```python
from build123d import *

# Parameters (mm, degrees)
SKETCH1_R           = 2
BOSS_EXTRUDE1_DEPTH = 10.8
SKETCH2_R           = 1.7
BOSS_EXTRUDE2_DEPTH = 0.6
SKETCH3_R           = 2
BOSS_EXTRUDE3_DEPTH = 1.6
CHAMFER1_SIZE       = 0.5


with BuildPart() as part:
    # Sketch1 → Boss-Extrude1 (new body)
    with BuildSketch(Plane.XY):
        with Locations(Location((0, 0, 0), (0, 0, 180))):
            Circle(SKETCH1_R)
    extrude(amount=BOSS_EXTRUDE1_DEPTH)

    # Sketch2 → Boss-Extrude2 (add)
    with BuildSketch(Plane.XY.offset(10.8)):
        Circle(SKETCH2_R)
    extrude(amount=BOSS_EXTRUDE2_DEPTH)

    # Sketch3 → Boss-Extrude3 (add)
    with BuildSketch(Plane.XY.offset(11.4)):
        with Locations(Location((0, 0, 0), (0, 0, 180))):
            Circle(SKETCH3_R)
    extrude(amount=BOSS_EXTRUDE3_DEPTH)

    # Chamfer1
    chamfer1_edges = [part.edges().sort_by_distance(p)[0] for p in [
        (2, 0, 13),
    ]]
    chamfer(chamfer1_edges, length=CHAMFER1_SIZE)


solid = part.part
```
CAD build for the part. Positions are in the model's coordinates, mm. Coordinates: 2 decimals unless noted, no trailing zeros. Write each loop counter-clockwise with the first axis right and the second up, starting at its lowest first coordinate (ties: lowest second). Pieces come first, ordered by that corner, then holes.
(1) Two-plate mould, pull along Z, no slides. Class faces 1 (the face through (0, 0, 0)), 2 (the face through (0, 2, 5)), 3 (the face through (-0.37, -1.66, 11.1)), 4 (the face through (0, 0, 13)): +Z half, -Z half, draft (parallel to the pull), parting line (faces both ways), or undercut.
(2) Flat gauge pins, fed straight in: pin 1 (2 mm diameter, centred on x = -0.5, y = -0.5, fed in from -Z); pin 2 (1.5 mm diameter, centred on y = 1, z = 9, fed in from +X). Where does each tip first touch, or does it go through?
(3) Drill centre lines: probe 1 along Z at (x, y) = (-0.9, 1.6); probe 2 along Y at (x, z) = (-1.8, 11.75); probe 3 along X at (y, z) = (1.6, 1). Where is each one in solid material? Low to high.
(4) Cut at A-A, the plane z = 1.5. List the corners of the cut face in (x, y), and give its area (3 significant figures).
Geometry says:
1. face 1: -Z half
1. face 2: draft
1. face 3: undercut
1. face 4: +Z half
2. pin 1: stops at z = 0
2. pin 2: stops at x = 1.98
3. probe 1: z = 0 to 10.8, 11.4 to 12.66
3. probe 2: y = -0.87 to 0.87
3. probe 3: x = -1.2 to 1.2
4. outline: circle Ø4 at (0, 0)
4. area: 12.6 mm2
